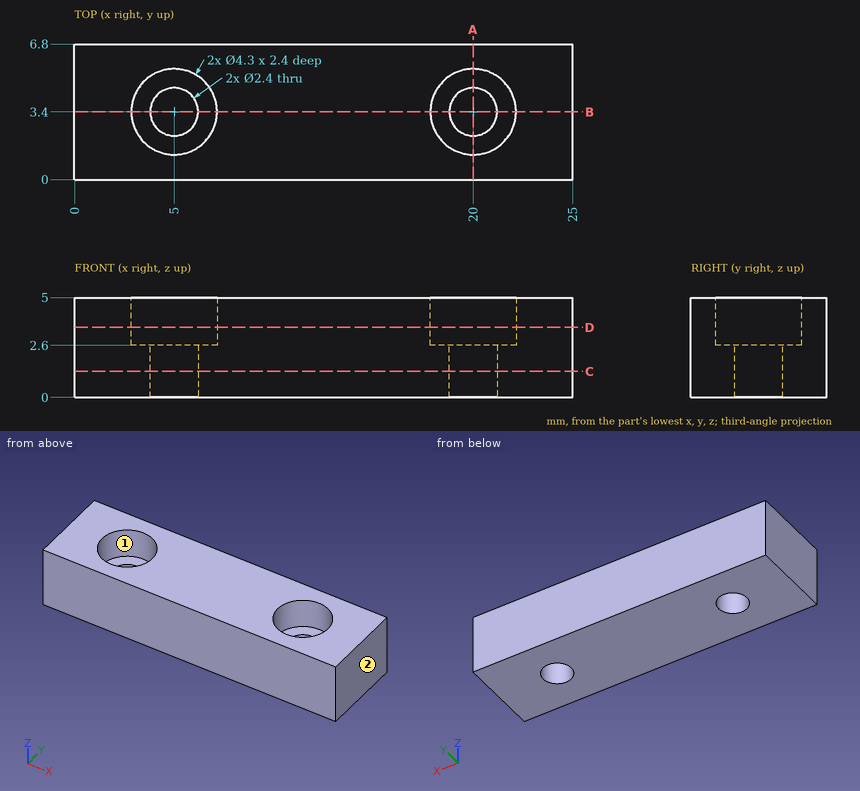
Source: three-view drawing plus pictorial views. Frame: mm from the lowest corner of the part. A direction names the side the tool comes from. Coordinates: 2 decimals unless noted, no trailing zeros. Order: outer loops, then holes, each group sorted by start corner. A loop starts at its lowest first (then second) coordinate and runs counter-clockwise, first axis right, second up. Notation, with made-up numbers: M -28.75,-29.75 L 5.25,-29.75 A16 cw 5.25,-5.75 Z; hole C -10,81 d11. An arc over 180 degrees is marked long. One line per question, with ' | ' between items.
Item 1: Reachability of the marked faces 1 and 2 from +Z, -Z, +X, -X, +Y, -Y: full face, straight path, thin tool, end or side. Return the list, or none.
Geometry results:
face 1: +Z | face 2: +Z, -Z, +X, +Y, -Y
Item 2: Section D-D (z = 3.5). Output: boundary loops of the cut face in (x, y).
Geometry results:
outline: M 0,0 L 25,0 L 25,6.8 L 0,6.8 Z; hole C 5,3.4 d4.3; hole C 20,3.4 d4.3
Item 3: Section B-B (y = 3.4). Output: boundary loops of the cut face in (x, z), then the cut area to 3 significant figures.
Geometry results:
outline: M 0,0 L 3.8,0 L 3.8,2.6 L 2.85,2.6 L 2.85,5 L 0,5 Z; M 6.2,0 L 18.8,0 L 18.8,2.6 L 17.85,2.6 L 17.85,5 L 7.15,5 L 7.15,2.6 L 6.2,2.6 Z; M 21.2,0 L 25,0 L 25,5 L 22.15,5 L 22.15,2.6 L 21.2,2.6 Z | area: 91.9 mm^2
Item 4: Section A-A (x = 20). Output: boundary loops of the cut face in (y, z), then the cut area to 3 significant figures.
Geometry results:
outline: M 0,0 L 2.2,0 L 2.2,2.6 L 1.25,2.6 L 1.25,5 L 0,5 Z; M 4.6,0 L 6.8,0 L 6.8,5 L 5.55,5 L 5.55,2.6 L 4.6,2.6 Z | area: 17.4 mm^2
Item 5: Pin query (flat end, axial travel): pin 1 (4 mm diameter, centred on x = 20, y = 3.4, fed in from +Z). Return the tip coordinate at first contact, or that it passes through.
Geometry results:
pin 1: stops at z = 2.6
Item 6: Ray query, line 1 along X through (y, z) = (3.5, 3.35); line 2 along Y through (x, z) = (20, 3.9); line 3 along X through (y, z) = (5.25, 3.85). Return the intervals inside material, ascending.
Geometry results:
line 1: x = 0 to 2.85, 7.15 to 17.85, 22.15 to 25 | line 2: y = 0 to 1.25, 5.55 to 6.8 | line 3: x = 0 to 3.9, 6.1 to 18.9, 21.1 to 25
Item 7: Section C-C (z = 1.3). Output: boundary loops of the cut face in (x, y).
Geometry results:
outline: M 0,0 L 25,0 L 25,6.8 L 0,6.8 Z; hole C 5,3.4 d2.4; hole C 20,3.4 d2.4
